```python
from build123d import *

# Parameters (mm, degrees)
EXTRUDE_1_DEPTH     = 2
SKETCH_2_R          = 5
CUT_EXTRUDE_1_DEPTH = 10


with BuildPart() as part:
    # 草图1 → 凸台-拉伸1 (new body)
    with BuildSketch(Plane.XY):
        Polygon((270.4264573, -50.479352133), (-291.276967283, -50.479352133), (-334.231201576, -307.163734724), (196.869820345, -490.036482017), align=None)
    extrude(amount=EXTRUDE_1_DEPTH)

    # 草图2 → 切除-拉伸1 (cut)
    with BuildSketch(Plane.XY.offset(2)):
        with Locations((-208.545453815, -102.175560394)):
            Circle(SKETCH_2_R)
        with Locations((-239.079260899, -284.638396678)):
            Circle(SKETCH_2_R)
        with Locations((-38.883807069, -224.353404635)):
            Circle(SKETCH_2_R)
        with Locations((130.777839678, -346.531248876)):
            Circle(SKETCH_2_R)
        with Locations((161.311646762, -164.068412591)):
            Circle(SKETCH_2_R)
    extrude(amount=-CUT_EXTRUDE_1_DEPTH, mode=Mode.SUBTRACT)


solid = part.part
```
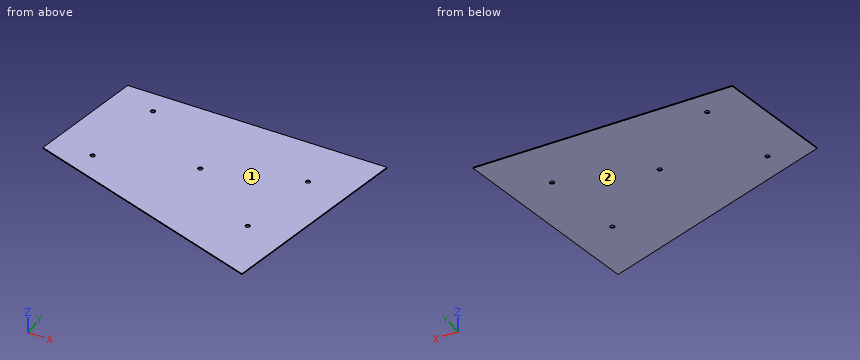
Can you work these out from the model? Positions are in its coordinate system, mm. Face numbers are marked on the shaded views. Coordinates: 2 decimals unless noted, no trailing zeros. Order: outer loops, then holes, each group sorted by start corner. A loop starts at its lowest first (then second) coordinate and runs counter-clockwise, first axis right, second up. Notation, with made-up numbers: (54.5, 20) - (75.5, 20) arc R17 ccw to (75.5, 28) - close; hole circle Ø5 at (57, 80). An arc over 180 degrees is marked (long way). Answer in a Markdown table with one row per item.
1. If I drill on line 1 along X through (y, z) = (-223.5, 0.6); line 2 along X through (y, z) = (-133, 1.95); line 3 along X through (y, z) = (-241, 1.35), over which ranges is the centre line in solid material (lowest first)?
Reply:
| item | result |
|---|---|
| line 1 | x = -320.23 to -43.81, -33.96 to 241.47 |
| line 2 | x = -305.09 to 256.62 |
| line 3 | x = -323.16 to 238.54 |
2. If we mould it in two halves opening along Z, with no side actions, what happens to the marked faces 1 and 2? For each: pulls with the +Z half, pulls with the -Z half, needs draft (parallel to the pull), parting line crosses it, or undercut.
Reply:
| item | result |
|---|---|
| face 1 | pulls with the +Z half |
| face 2 | pulls with the -Z half |
3. Suppose I cut it at B-B (x = -252.5). Please give me the cut outline in (y, z).
Reply:
| item | result |
|---|---|
| outline | (-335.31, 0) - (-50.48, 0) - (-50.48, 2) - (-335.31, 2) - close |
4. Suppose I cut it at A-A (z = 1.55). Please give me the cut outline in (x, y).
Reply:
| item | result |
|---|---|
| outline | (-334.23, -307.16) - (196.87, -490.04) - (270.43, -50.48) - (-291.28, -50.48) - close; hole circle Ø10 at (-239.08, -284.64); hole circle Ø10 at (-208.55, -102.18); hole circle Ø10 at (-38.88, -224.35); hole circle Ø10 at (130.78, -346.53); hole circle Ø10 at (161.31, -164.07) |
5. Suppose I cut it at C-C (y = -362). Please give me the cut outline in (x, z), and give its area (3 significant figures).
Reply:
| item | result |
|---|---|
| outline | (-174.98, 0) - (218.3, 0) - (218.3, 2) - (-174.98, 2) - close |
| area | 787 mm^2 |
